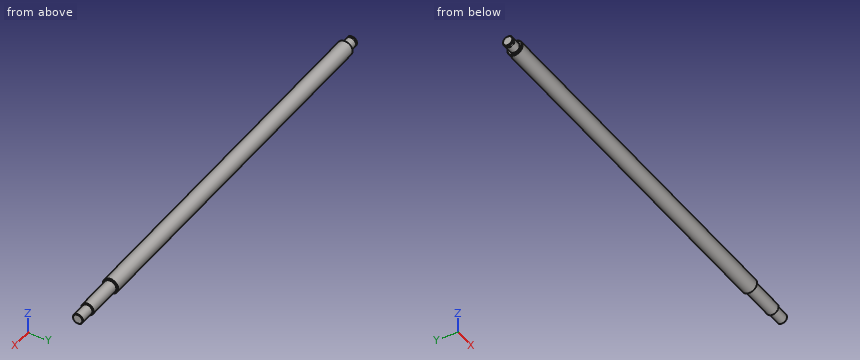
from build123d import *


with BuildPart() as part:
    # Sketch1 → Revolve1 (revolve)
    with BuildSketch(Plane.XY, mode=Mode.PRIVATE) as revolve1_sk:
        with BuildLine():
            Line((1.85, 5), (1.85, 4.8))
            Line((1.85, 4.8), (3, 4.8))
            Line((3, 4.8), (3, 5))
            Line((3, 5), (10.7, 5))
            ThreePointArc((10.7, 5), (10.912132034, 5.087867966), (11, 5.3))
            Line((11, 5.3), (11, 7))
            Line((11, 7), (11.5, 7.5))
            Line((11.5, 7.5), (378.5, 7.5))
            Line((378.5, 7.5), (379, 7))
            Line((379, 7), (379, 6.3))
            ThreePointArc((379, 6.3), (379.087867966, 6.087867966), (379.3, 6))
            Line((379.3, 6), (414.5, 6))
            Line((414.5, 6), (415, 5.5))
            Line((415, 5.5), (415, 5.2))
            ThreePointArc((415, 5.2), (415.058578644, 5.058578644), (415.2, 5))
            Line((415.2, 5), (429.5, 5))
            Line((429.5, 5), (430, 4.5))
            Line((430, 4.5), (430, 0))
            Line((430, 0), (0, 0))
            Line((0, 0), (0, 4.5))
            Line((0, 4.5), (0.5, 5))
            Line((0.5, 5), (1.85, 5))
        make_face()
    revolve(revolve1_sk.sketch.rotate(Axis((-7.5, 0, 0), (1, 0, 0)), 90), axis=Axis((-7.5, 0, 0), (1, 0, 0)))


solid = part.part
Input: part model. Units: mm. Frame: model coordinates. Round coordinates to 2 decimals unless told otherwise and drop trailing zeros. Order: outer loops, then holes, each group sorted by start corner. A loop starts at its lowest first (then second) coordinate and runs counter-clockwise, first axis right, second up.
1. Pin query (flat end, axial travel): P1, Ø5, axis at x = 321.5, z = -4.5, coming from the -Y side; P2, Ø5, axis at y = 6, z = 6, coming from the -X side; P3, Ø2, axis at x = 262, y = -5.5, coming from the +Z side. Return the tip coordinate at first contact, or that it passes through.
The answers:
P1: stops at y = -7.23
P2: stops at x = 11
P3: stops at z = 6
2. Cut plane A-A, the plane x = 64. Output: boundary loops of the cut face in (y, z), then the cut area to 3 significant figures.
The answers:
outline: circle Ø15 at (0, 0)
area: 177 mm2
3. Material intervals for line 1 (X direction, y = -4, z = 3.5); line 2 (Y direction, x = 99.5, z = -4); line 3 (Y direction, x = 398, z = 0), sorted ascending.
The answers:
line 1: x = 11 to 415
line 2: y = -6.34 to 6.34
line 3: y = -6 to 6
